```python
from build123d import *


with BuildPart() as part:
    # Sketch1 → Revolve1 (revolve)
    with BuildSketch(Plane.XY, mode=Mode.PRIVATE) as revolve1_sk:
        with BuildLine():
            Line((0, 27.5), (0, 46))
            ThreePointArc((0, 46), (3, 47.354248689), (6, 46))
            Line((6, 46), (27.497518595, 43.85024814))
            ThreePointArc((27.497518595, 43.85024814), (30.707262668, 42.230088793), (32, 38.875062189))
            Line((32, 38.875062189), (32, 38))
            Line((32, 38), (22, 38))
            Line((22, 38), (22, 36))
            Line((22, 36), (10, 36))
            Line((10, 36), (10, 27.5))
            Line((10, 27.5), (7.4, 27.5))
            Line((7.4, 27.5), (7.4, 30.35))
            Line((7.4, 30.35), (2.6, 30.35))
            Line((2.6, 30.35), (2.6, 27.5))
            Line((2.6, 27.5), (0, 27.5))
        make_face()
    revolve(revolve1_sk.sketch.rotate(Axis((-44.681900546, 0, 0), (1, 0, 0)), 90), axis=Axis((-44.681900546, 0, 0), (1, 0, 0)))


solid = part.part
```
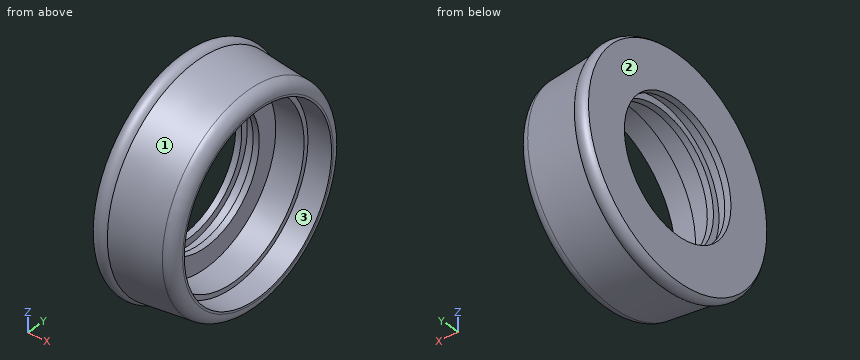
Check sheet for the modelled part. Datum: model origin and axes. Units: mm. Face numbers are marked on the shaded views. Give positions to 0.01 mm unless a question says otherwise; leave off trailing zeros. Order: outer loops, then holes, each group sorted by start corner. A loop starts at its lowest first (then second) coordinate and runs counter-clockwise, first axis right, second up. Notation, with made-up numbers: M 34,-12.5 L 47,-12.5 A36 ccw 47,25.5 Z; hole C -12,82.25 d2. An arc over 180 degrees is marked long. Answer in a Markdown table with one row per item. Add a question column.
Q1. Sectioned sample at D-D, the plane x = 19.5. Record the boundary of the cut face in (y, z).
Q2. Thickness scan on L1, parallel to Y at x = 21.5, z = -2.5; L2, parallel to Y at x = 9.5, z = -4.5; L3, parallel to Z at x = 23, y = -31. Record the ranges inside material, lowest first.
Q3. Sectioned sample at C-C, the plane x = 26. Record the boundary of the cut face in (y, z), and give its area (3 significant figures).
Q4. Sectioned sample at A-A, the plane z = 0. Record the boundary of the cut face in (x, y).
Q5. Release check for a two-part mould opening along Y. For the marked faces 1, 2 and 3 record: released by +Y, released by -Y, zero draft, split by the parting line, or undercut.
Q6. Gauge pin test, flat ends, axial feed: pin 1 Ø1.5 at (y, z) = (25.5, -28) entering from -X; pin 2 Ø10 at (x, z) = (6.5, -14) entering from +Y; pin 3 Ø18 at (y, z) = (-0.5, -14) entering from -X; pin 4 Ø5 at (x, z) = (10.5, 37) entering from +Y. Record the tip position at first contact, or that the pin passes through.
Verdict:
| question | item | result |
|---|---|---|
| 1 | outline | C 0,0 d89.3; hole C 0,0 d72 |
| 2 | L1 | -44.38 to -35.91, 35.91 to 44.38 |
| 2 | L2 | -45.43 to -27.13, 27.13 to 45.43 |
| 2 | L3 | -31.65 to -21.98, 21.98 to 31.65 |
| 3 | outline | C 0,0 d88; hole C 0,0 d76 |
| 3 | area | 1,550 mm² |
| 4 | outline | M 0,-46 A4 ccw 6,-46 L 27.5,-43.85 A5 ccw 32,-38.88 L 32,-38 L 22,-38 L 22,-36 L 10,-36 L 10,-27.5 L 7.4,-27.5 L 7.4,-30.35 L 2.6,-30.35 L 2.6,-27.5 L 0,-27.5 Z; M 0,27.5 L 2.6,27.5 L 2.6,30.35 L 7.4,30.35 L 7.4,27.5 L 10,27.5 L 10,36 L 22,36 L 22,38 L 32,38 L 32,38.88 A5 ccw 27.5,43.85 L 6,46 A4 ccw 0,46 Z |
| 5 | face 1 | split by the parting line |
| 5 | face 2 | zero draft |
| 5 | face 3 | undercut |
| 6 | pin 1 | x = 0 |
| 6 | pin 2 | y = 46.26 |
| 6 | pin 3 | through |
| 6 | pin 4 | y = 29.77 |
